Study the drawing (mm; zero at the part's minimum x, y, z) and answer. Coordinates: 2 decimals unless noted, no trailing zeros. Order: outer loops, then holes, each group sorted by start corner. A loop starts at its lowest first (then second) coordinate and runs counter-clockwise, first axis right, second up. Notation, with made-up numbers: (-11, -39.5) -> (1, -39.5) arc R26 cw to (1, -18.5) -> close; hole circle Ø9 at (14, 15.25). An arc over 180 degrees is marked (long way). One line per question, with ' | ' between items.
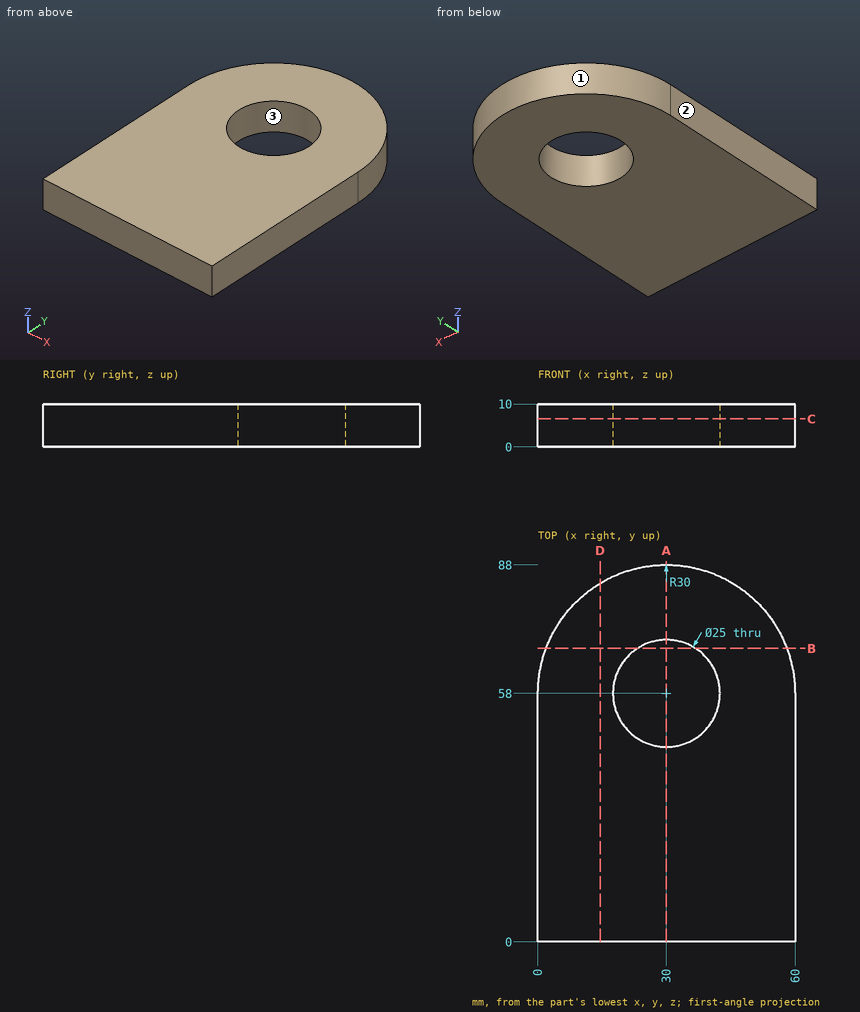
Item 1: Section C-C, the plane z = 6.5 is taken. Give the vertices of the cut face in (x, y), plus the area to 3 significant figures.
Computed values:
outline: (0, 0) -> (60, 0) -> (60, 58) arc R30 ccw to (0, 58) -> close; hole circle Ø25 at (30, 58) | area: 4,400 mm^2
Item 2: Each of these flat-tipped pins is pushed along its axis until it touches: pin 1 Ø15 at (x, y) = (30, 58) entering from -Z; pin 2 Ø2 at (x, z) = (48.5, 8) entering from +Y; pin 3 Ø6 at (y, z) = (31.5, 6.5) entering from -X. Where does it stop, or does it pass through?
Computed values:
pin 1: passes through | pin 2: stops at y = 82.37 | pin 3: stops at x = 0
Item 3: Find the intervals of material crossed by L1, parallel to Y at x = 30, z = 6.25; L2, parallel to X at y = 64, z = 1.5; L3, parallel to Y at x = 24.5, z = 9, in increasing order.
Computed values:
L1: y = 0 to 45.5, 70.5 to 88 | L2: x = 0.61 to 19.03, 40.97 to 59.39 | L3: y = 0 to 46.78, 69.22 to 87.49
Item 4: Section D-D, the plane x = 14.5 is taken. Give the vertices of the cut face in (y, z).
Computed values:
outline: (0, 0) -> (83.69, 0) -> (83.69, 10) -> (0, 10) -> close
Item 5: Determine the mould class of the marked faces 1, 2 and 3 for opening direction Y: pulls with the +Y half, pulls with the -Y half, needs draft (parallel to the pull), parting line crosses it, or undercut.
Computed values:
face 1: pulls with the +Y half | face 2: needs draft | face 3: undercut
Item 6: Section B-B, the plane y = 68.5 is taken. Give the vertices of the cut face in (x, z), plus the area to 3 significant figures.
Computed values:
outline: (1.9, 0) -> (23.22, 0) -> (23.22, 10) -> (1.9, 10) -> close; (36.78, 0) -> (58.1, 0) -> (58.1, 10) -> (36.78, 10) -> close | area: 426 mm^2
Item 7: Section A-A, the plane x = 30 is taken. Give the vertices of the cut face in (y, z).
Computed values:
outline: (0, 0) -> (45.5, 0) -> (45.5, 10) -> (0, 10) -> close; (70.5, 0) -> (88, 0) -> (88, 10) -> (70.5, 10) -> close
